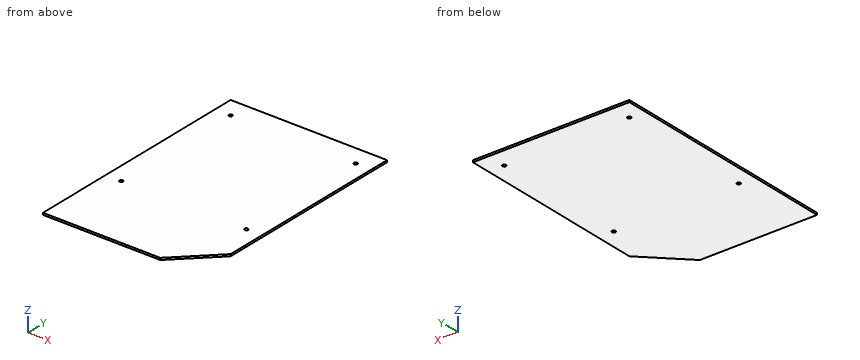
from build123d import *

# Parameters (mm, degrees)
SKETCH_1_W          = 400
SKETCH_1_H          = 600
EXTRUDE_1_DEPTH     = 5
SKETCH_2_R          = 4.5
CUT_EXTRUDE_1_DEPTH = 361.589794642
CHAMFER_1_SIZE      = 100


with BuildPart() as part:
    # 草图1 → 凸台-拉伸1 (new body)
    with BuildSketch(Plane.XY):
        Rectangle(SKETCH_1_W, SKETCH_1_H)
    extrude(amount=EXTRUDE_1_DEPTH)

    # 草图2 → 切除-拉伸1 (cut, through all)
    with BuildSketch(Plane.XY.offset(5)):
        with Locations((-160, 250)):
            Circle(SKETCH_2_R)
        with Locations((160, 250)):
            Circle(SKETCH_2_R)
        with Locations((160, -100)):
            Circle(SKETCH_2_R)
        with Locations((-160, -100)):
            Circle(SKETCH_2_R)
    extrude(amount=-CUT_EXTRUDE_1_DEPTH, mode=Mode.SUBTRACT)

    # 倒角1
    chamfer_1_edges = [part.edges().sort_by_distance(p)[0] for p in [
        (200, -300, 2.5),
    ]]
    chamfer(chamfer_1_edges, length=CHAMFER_1_SIZE)


solid = part.part
The listing builds one solid part. Answer for the finished solid, in the listing's coordinates (mm). Give positions to 0.01 mm unless a question says otherwise; leave off trailing zeros. Loops run counter-clockwise (first coordinate to the right, second up) from the corner with the lowest first, then second, coordinate; pieces in that order, holes last. Notation, with made-up numbers: (54.25, -26.5) - (83.25, -26.5) arc R16 cw to (83.25, -2.5) - close; hole circle Ø7 at (1, 59). An arc over 180 degrees is marked (long way). Write each question's results on one line, items separated by ' | '.
1. Consider probe 1 along Y at (x, z) = (-160, 4); probe 2 along Y at (x, z) = (160, 3.75); probe 3 along Y at (x, z) = (152, 0.55). Determine where each line is inside the solid, lowest interval first. Write a range as from..to.
Resolved:
probe 1: y = -300..-104.5, -95.5..245.5, 254.5..300 | probe 2: y = -240..-104.5, -95.5..245.5, 254.5..300 | probe 3: y = -248..300
2. A flat-ended cylindrical pin translates along its axis: P1, Ø3, axis at y = -213, z = 3.5, coming from the +X side. Find the tip coordinate at first contact, or state that the pin passes through.
Resolved:
P1: stops at x = 188.5
3. Find section A-A, the plane z = 2. Write down the section's boundary in (x, y), then the cut area to 3 significant figures.
Resolved:
outline: (-200, -300) - (100, -300) - (200, -200) - (200, 300) - (-200, 300) - close; hole circle Ø9 at (-160, -100); hole circle Ø9 at (-160, 250); hole circle Ø9 at (160, -100); hole circle Ø9 at (160, 250) | area: 235,000 mm^2
